```python
from build123d import *

# Parameters (mm, degrees)
HUB_TUBE_SKETCH_50_25_R   = 25
HUB_TUBE_SKETCH_50_25_R_2 = 12.5
HUB_TUBE_50_25_X35_DEPTH  = 17.5
ARM_50_DEPTH              = 25
TOP_NOTCH_CUT_DEPTH       = 111.509908397
CROSS_HOLE_SKETCH_10_R    = 5
CROSS_HOLE_10_DEPTH       = 101.657736852
BORE_CLEARANCE_CUT_DEPTH  = 108.931611768


with BuildPart() as part:
    # Hub Tube Sketch Ø50-Ø25 → Hub Tube Ø50-Ø25 x35 (new, symmetric)
    with BuildSketch(Plane.XY):
        Circle(HUB_TUBE_SKETCH_50_25_R)
        Circle(HUB_TUBE_SKETCH_50_25_R_2, mode=Mode.SUBTRACT)
    extrude(amount=HUB_TUBE_50_25_X35_DEPTH, both=True)

    # Arm Profile Sketch → Arm 50 (add, symmetric)
    with BuildSketch(Plane(origin=(0, 0, 0), x_dir=(1, 0, 0), z_dir=(0, 1, 0))):
        Polygon((3.520588359, 7.5), (-25, 7.5), (-50, 7.5), (-94.271090497, -15.73941794), (-86.771090497, -28.729798997), (-50, -7.5), (-25, -7.5), (3.520588359, -7.5), align=None)
    extrude(amount=ARM_50_DEPTH, both=True)

    # Top Notch Sketch → Top Notch Cut (cut, through all)
    with BuildSketch(Plane(origin=(0, 25, 0), x_dir=(1, 0, 0), z_dir=(0, 1, 0))):
        Polygon((-76.562654298, -6.443650764), (-74.238712504, -10.870759814), (-65.384494405, -6.222876226), (-67.708436199, -1.795767176), align=None)
    extrude(amount=-TOP_NOTCH_CUT_DEPTH, mode=Mode.SUBTRACT)

    # Cross Hole Sketch Ø10 → Cross Hole Ø10 (cut, through all)
    with BuildSketch(Plane(origin=(-13.887914048, 0, -26.456475856), x_dir=(-0.8854218099422658, 0, 0.46478835880275915), z_dir=(-0.46478835880275915, 0, -0.8854218099422658))):
        with Locations((80.785177806, 0)):
            Circle(CROSS_HOLE_SKETCH_10_R)
    extrude(amount=-CROSS_HOLE_10_DEPTH, mode=Mode.SUBTRACT)

    # Bore Clearance Sketch → Bore Clearance Cut (cut, through all)
    with BuildSketch(Plane(origin=(0, 0, -17.5), x_dir=(-1, 0, 0), z_dir=(0, 0, -1))):
        with BuildLine():
            Line((-3.520588359, 11.993975888), (-3.520588359, -11.993975888))
            ThreePointArc((-3.520588359, -11.993975888), (12.5, 0), (-3.520588359, 11.993975888))
        make_face()
    extrude(amount=-BORE_CLEARANCE_CUT_DEPTH, mode=Mode.SUBTRACT)


solid = part.part
```
Verification items for the finished model (mm, model axes). A direction names the side the tool comes from. Give positions to 0.01 mm unless a question says otherwise; leave off trailing zeros. Order: outer loops, then holes, each group sorted by start corner. A loop starts at its lowest first (then second) coordinate and runs counter-clockwise, first axis right, second up. Notation, with made-up numbers: M 8.5,8 L 55.5,8 A12 ccw 55.5,18 Z; hole C -30,68 d3. An arc over 180 degrees is marked long. Answer in a Markdown table with one row per item. Add a question column.
Item 1: Gauge pin test, flat ends, axial feed: pin 1 (15 mm diameter, centred on x = 0, y = 0, fed in from -Z); pin 2 (4 mm diameter, centred on x = 6, z = 3, fed in from +Y); pin 3 (5 mm diameter, centred on y = 11, z = -2, fed in from +X); pin 4 (12 mm diameter, centred on y = -1, z = 19.5, fed in from -X). Record the tip position at first contact, or that the pin passes through.
Item 2: Tool access check on faces 1 (the flat face through (-75.417, 0.35, 8.626)), 2 (the flat face through (-66.53, 0.35, 4.04)), 3 (the flat face through (-11.5, 5.9, 17.5)), 4 (the flat face through (-68.64, 0.35, 18.26)). Record the directions out of +Z, -Z, +X, -X, +Y, -Y that give a thin tool (end or side, any length) a straight path to the whole face; none if there is none.
Item 3: Scan lines: probe 1 along X at (y, z) = (0, 7); probe 2 along X at (y, z) = (0, -9). Record each from-to range of solid material in increasing order. Write a range as from..to.
Item 4: Mould release check, pull along Z, two halves, no side actions. Record for faces 5 (the flat face through (-69.874, 0.35, 8.579)), 6 (the flat face through (-36, 0, 7.5)), 7 (the flat face through (-36, 0, -7.5)), 8 (the cylindrical face through (11.923, 3.755, -0.245)): released by +Z, released by -Z, zero draft, split by the parting line, or undercut.
Item 5: Section check C-C, the plane y = 0. Enter the section's corners in (x, z), and give its area (3 significant figures).
Item 6: Section check D-D, the plane x = -29. Enter the section's corners in (y, z).
Item 7: Section check A-A, the plane y = -10.5. Enter the section's corners in (x, z), and give its area (3 significant figures).
Item 8: Section check B-B, the plane z = -1. Enter the section's corners in (x, y), and give its area (3 significant figures).
Filled sheet:
| question | item | result |
|---|---|---|
| 1 | pin 1 | passes through |
| 1 | pin 2 | stops at y = 24.68 |
| 1 | pin 3 | stops at x = 23.51 |
| 1 | pin 4 | stops at x = -94.27 |
| 2 | face 1 | -Z, +Y, -Y |
| 2 | face 2 | -X, +Y, -Y |
| 2 | face 3 | +Z, +X, +Y, -Y |
| 2 | face 4 | +Z, +Y, -Y |
| 3 | probe 1 | x = -77.62..-76.27, -66.86..-12.5, 12.5..25 |
| 3 | probe 2 | x = -25..-12.5, 12.5..25 |
| 4 | face 5 | undercut |
| 4 | face 6 | released by +Z |
| 4 | face 7 | released by -Z |
| 4 | face 8 | zero draft |
| 5 | outline | M -94.27,15.74 L -89.84,13.42 L -82.96,26.53 L -86.77,28.73 Z; M -80.99,8.77 L -76.56,6.44 L -74.24,10.87 L -65.38,6.22 L -67.71,1.8 L -50,-7.5 L -25,-7.5 L -25,-17.5 L -12.5,-17.5 L -12.5,17.5 L -25,17.5 L -25,7.5 L -50,7.5 L -74.29,21.53 Z; M 12.5,-17.5 L 25,-17.5 L 25,17.5 L 12.5,17.5 Z |
| 5 | area | 1,700 mm^2 |
| 6 | outline | M -25,-7.5 L 25,-7.5 L 25,7.5 L -25,7.5 Z |
| 7 | outline | M -94.27,15.74 L -76.56,6.44 L -74.24,10.87 L -65.38,6.22 L -67.71,1.8 L -50,-7.5 L -22.69,-7.5 L -22.69,-17.5 L -6.78,-17.5 L -6.78,17.5 L -22.69,17.5 L -22.69,7.5 L -50,7.5 L -86.77,28.73 Z; M 6.78,-17.5 L 22.69,-17.5 L 22.69,17.5 L 6.78,17.5 Z |
| 7 | area | 2,120 mm^2 |
| 8 | outline | M -62.38,-25 L 3.52,-25 L 3.52,-24.75 A25 ccw 3.52,24.75 L 3.52,25 L -62.38,25 Z; hole C 0,0 d25 |
| 8 | area | 3,610 mm^2 |
